Input: part model. Units: mm. Frame: model coordinates. A direction names the side the tool comes from. Coordinates: 2 decimals unless noted, no trailing zeros. Loops run counter-clockwise (first coordinate to the right, second up) from the corner with the lowest first, then second, coordinate; pieces in that order, holes last. Notation, with made-up numbers: (42.25, 4) -> (92.25, 4) arc R14 cw to (92.25, 13) -> close; hole circle Ø10 at (85, -16.75). An arc over 180 degrees is marked (long way). Answer as a JSON object with one key per item and string values.
from build123d import *

# Parameters (mm, degrees)
BRACKET_PROFILE_SKETCH_R = 15
L_BRACKET_BODY_DEPTH     = 11.5
SLOT_CUT_SKETCH_W        = 16
SLOT_CUT_SKETCH_H        = 12
SLOT_CUT_DEPTH           = 63
END_HOLE_SKETCH_R        = 3
END_HOLE_DEPTH           = 63


with BuildPart() as part:
    # Bracket Profile Sketch → L-Bracket Body (new, symmetric)
    with BuildSketch(Plane.XY):
        with BuildLine():
            Line((73, 3), (73, -124))
            Line((73, -124), (45, -124))
            Line((45, -124), (45, -35))
            ThreePointArc((45, -35), (42.363961031, -28.636038969), (36, -26))
            Line((36, -26), (-23, -26))
            Line((-23, -26), (-23, 26))
            Line((-23, 26), (50, 26))
            ThreePointArc((50, 26), (66.263455967, 19.263455967), (73, 3))
        make_face()
        Circle(BRACKET_PROFILE_SKETCH_R, mode=Mode.SUBTRACT)
    extrude(amount=L_BRACKET_BODY_DEPTH, both=True)

    # Slot Cut Sketch → Slot Cut (cut)
    with BuildSketch(Plane(origin=(0, 26, 0), x_dir=(1, 0, 0), z_dir=(0, 1, 0))):
        with Locations((-15, 0)):
            Rectangle(SLOT_CUT_SKETCH_W, SLOT_CUT_SKETCH_H)
    extrude(amount=-SLOT_CUT_DEPTH, mode=Mode.SUBTRACT)

    # End Hole Sketch → End Hole (cut)
    with BuildSketch(Plane(origin=(73, 0, 0), x_dir=(0, 0, -1), z_dir=(1, 0, 0))):
        with Locations(Location((0, -112, 0), (0, 0, 90))):
            Circle(END_HOLE_SKETCH_R)
    extrude(amount=-END_HOLE_DEPTH, mode=Mode.SUBTRACT)


solid = part.part
1. Section query B-B (z = 0). Return loops of the section in (x, y), plus the area to 3 significant figures.
Reply:
{"outline": "(-7, -26) -> (36, -26) arc R9 cw to (45, -35) -> (45, -109) -> (73, -109) -> (73, 3) arc R23 ccw to (50, 26) -> (-7, 26) -> (-7, 13.27) arc R15 cw (long way) to (-7, -13.27) -> close; (45, -124) -> (73, -124) -> (73, -115) -> (45, -115) -> close", "area": "6,080 mm2"}
2. Line query: line 1 along Z through (x, y) = (64.25, -112); line 2 along X through (y, z) = (0, 7); line 3 along Y through (x, z) = (0, 0.5). Output: solid intervals per line, ascending.
Reply:
{"line 1": "z = -11.5 to -3, 3 to 11.5", "line 2": "x = -23 to -15, 15 to 73", "line 3": "y = -26 to -15, 15 to 26"}
3. Section query D-D (x = 0). Return loops of the section in (y, z), plus the area to 3 significant figures.
Reply:
{"outline": "(-26, -11.5) -> (-15, -11.5) -> (-15, 11.5) -> (-26, 11.5) -> close; (15, -11.5) -> (26, -11.5) -> (26, 11.5) -> (15, 11.5) -> close", "area": "506 mm2"}
4. Section query C-C (y = -112). Return loops of the section in (x, z).
Reply:
{"outline": "(45, -11.5) -> (73, -11.5) -> (73, -3) -> (45, -3) -> close; (45, 3) -> (73, 3) -> (73, 11.5) -> (45, 11.5) -> close"}
5. Access query for faces 4 (the face through (59, -124, 0)), 5 (the face through (-7, -20, 0)), 6 (the face through (45, -80, 0)). Directions: +Z, -Z, +X, -X, +Y, -Y. A direction counts if a zero-diameter tool reaches every point of the face in a straight line with its end or side. Return the directions, or none.
Reply:
{"face 4": "+Z, -Z, +X, -X, -Y", "face 5": "-X, +Y, -Y", "face 6": "+Z, -Z, -X, -Y"}
6. Pin query (flat end, axial travel): P1, Ø3, axis at y = -108, z = -9, coming from the -X side; P2, Ø6, axis at y = -18, z = -2, coming from the -X side; P3, Ø6, axis at x = 23, z = -6, coming from the -Y side. Return the tip coordinate at first contact, or that it passes through.
Reply:
{"P1": "stops at x = 45", "P2": "stops at x = -7", "P3": "stops at y = -26"}
7. Section query A-A (y = 0). Return loops of the section in (x, z).
Reply:
{"outline": "(-23, -11.5) -> (-15, -11.5) -> (-15, -6) -> (-23, -6) -> close; (-23, 6) -> (-15, 6) -> (-15, 11.5) -> (-23, 11.5) -> close; (15, -11.5) -> (73, -11.5) -> (73, 11.5) -> (15, 11.5) -> close"}
8. Mould query, pull axis Y, two halves, no side actions, for faces 1 (the face through (47, -31, 11.5)), 2 (the face through (7, -26, 0)), 3 (the face through (14.307, 4.506, -0.161)). Classes: pulls with the +Y half, pulls with the -Y half, needs draft (parallel to the pull), parting line crosses it, or undercut.
Reply:
{"face 1": "needs draft", "face 2": "pulls with the -Y half", "face 3": "undercut"}
